Read the model definition and answer for the solid it produces. Units are mm, in the model's axes. A direction names the side the tool comes from. Round coordinates to 2 decimals unless told otherwise and drop trailing zeros. Order: outer loops, then holes, each group sorted by start corner. A loop starts at its lowest first (then second) coordinate and runs counter-clockwise, first axis right, second up. Notation, with made-up numbers: (73.5, 46) - (111.5, 46) arc R20 cw to (111.5, 71) - close; hole circle Ø10 at (-30, 40.5). An arc over 180 degrees is marked (long way). Put each result on its own line as item: value. Start each with the question number.
Q1. Find the intervals of material crossed by line 1 along Y through (x, z) = (-12, 0.5); line 2 along Z through (x, y) = (0, 22); line 3 along Z through (x, y) = (-11.5, -2.5), in increasing order. Write a range as from..to.
Q2. Section D-D on x = -8.5 is taken. Give the vertices of the cut face in (y, z), then the cut area to 3 significant figures.
Q3. Section A-A on x = 0 is taken. Give the vertices of the cut face in (y, z), then the cut area to 4 significant figures.
Q4. Section C-C on y = -8 is taken. Give the vertices of the cut face in (x, z), then the cut area to 3 significant figures.
Q5. Each of these flat-tipped pins is pushed along its axis until it touches: pin 1 Ø2.5 at (y, z) = (-38.5, -8.5) entering from +X; pin 2 Ø1.5 at (x, y) = (4, -6) entering from +Z; pin 3 Ø3 at (x, z) = (-3, -16) entering from -Y. Where does it stop, or does it pass through?
Q6. Which of the six approach directions +Z, -Z, +X, -X, +Y, -Y give full straight-line access (tool end or side, diameter ignored) to faces 5 (the face through (-9, 15, 5)), 6 (the face through (-9, -15, -5)), 7 (the face through (0, -55, 0)), 8 (the face through (-0.1, 22.5, -8.8)), 9 (the face through (19.524, -0.21, -4.336))?
Q7. Section B-B on z = 0 is taken. Give the vertices of the cut face in (x, y), then the cut area to 3 significant figures.
Q8. For a pull along X with two mould halves and no side action, classify faces 1 (the face through (-2.5, -35, -9)), 2 (the face through (0, 55, 0)), 3 (the face through (0, 35, -7.5)), 4 (the face through (3.83, 34.72, 9.237)) as pulls with the +X half, pulls with the -X half, needs draft (parallel to the pull), parting line crosses it, or undercut.
from build123d import *

# Parameters (mm, degrees)
CUT_EXTRUDE1_DEPTH = 2.5


with BuildPart() as part:
    # Sketch1 → Revolve1 (revolve)
    with BuildSketch(Plane(origin=(0, 0, 0), x_dir=(0, 0, -1), z_dir=(1, 0, 0))):
        Polygon((0, 55), (-10, 55), (-10, 15), (-20, 15), (-20, -15), (-10, -15), (-10, -55), (0, -55), align=None)
    revolve(axis=Axis((0, 189.929754582, 0), (0, -1, 0)))

    # Sketch2 → Cut-Extrude1 (cut)
    with BuildSketch(Plane(origin=(0, 0, -10), x_dir=(-1, 0, 0), z_dir=(0, 0, -1))):
        with BuildLine():
            Line((2.5, 45), (2.5, 25))
            ThreePointArc((2.5, 25), (0, 22.5), (-2.5, 25))
            Line((-2.5, 25), (-2.5, 45))
            ThreePointArc((-2.5, 45), (0, 47.5), (2.5, 45))
        make_face()
    cut_extrude1 = extrude(amount=-CUT_EXTRUDE1_DEPTH, mode=Mode.SUBTRACT)

    # Mirror1: Cut-Extrude1 across plane
    add(cut_extrude1.mirror(Plane.ZX), mode=Mode.SUBTRACT)


solid = part.part
Findings:
1. line 1: -15..15
1. line 2: -10..10
1. line 3: -16.36..16.36
2. outline: (-55, -5.27) - (-15, -5.27) - (-15, -18.1) - (15, -18.1) - (15, -5.27) - (55, -5.27) - (55, 5.27) - (15, 5.27) - (15, 18.1) - (-15, 18.1) - (-15, 5.27) - (-55, 5.27) - close
2. area: 1,930 mm2
3. outline: (-55, -10) - (-47.5, -10) - (-47.5, -7.5) - (-22.5, -7.5) - (-22.5, -10) - (-15, -10) - (-15, -20) - (15, -20) - (15, -10) - (22.5, -10) - (22.5, -7.5) - (47.5, -7.5) - (47.5, -10) - (55, -10) - (55, 10) - (15, 10) - (15, 20) - (-15, 20) - (-15, 10) - (-55, 10) - close
3. area: 2,675 mm2
4. outline: circle Ø40 at (0, 0)
4. area: 1,260 mm2
5. pin 1: x = 6.89
5. pin 2: z = 19.73
5. pin 3: y = -15
6. face 5: +Y
6. face 6: -Y
6. face 7: +Z, -Z, +X, -X, -Y
6. face 8: -Z
6. face 9: +Y, -Y
7. outline: (-20, -15) - (-10, -15) - (-10, -55) - (10, -55) - (10, -15) - (20, -15) - (20, 15) - (10, 15) - (10, 55) - (-10, 55) - (-10, 15) - (-20, 15) - close
7. area: 2,800 mm2
8. face 1: undercut
8. face 2: needs draft
8. face 3: undercut
8. face 4: parting line crosses it
